For this review, take the finished solid that the model builds, in its own axes (mm). A direction names the side the tool comes from. Round coordinates to 2 decimals unless told otherwise and drop trailing zeros. Write each loop counter-clockwise with the first axis right and the second up, starting at its lowest first coordinate (ties: lowest second). Pieces come first, ordered by that corner, then holes. Notation, with made-up numbers: (85.25, 6.25) -> (123.25, 6.25) arc R19 cw to (123.25, 15.25) -> close; hole circle Ø6 at (-25, 18.5). An arc over 180 degrees is marked (long way). Write item = value, one per line. Start each with the question number.
```python
from build123d import *

# Parameters (mm, degrees)
CUT_EXTRUDE1_DEPTH = 2.5


with BuildPart() as part:
    # Sketch1 → Revolve1 (revolve)
    with BuildSketch(Plane(origin=(0, 0, 0), x_dir=(0, 0, -1), z_dir=(1, 0, 0)), mode=Mode.PRIVATE) as revolve1_sk:
        with BuildLine():
            Line((-1.633974596, 0), (-2.5, 1.5))
            Line((-2.5, 1.5), (-2.5, 3.8))
            ThreePointArc((-2.5, 3.8), (-2.441421356, 3.941421356), (-2.3, 4))
            Line((-2.3, 4), (-0.833333333, 4))
            Line((-0.833333333, 4), (-0.833333333, 3.6))
            Line((-0.833333333, 3.6), (-0.683333333, 3.6))
            Line((-0.683333333, 3.6), (-0.683333333, 4))
            Line((-0.683333333, 4), (0, 4))
            Line((0, 4), (0, 2.0095))
            Line((0, 2.0095), (0.4905, 2.5))
            Line((0.4905, 2.5), (3.3095, 2.5))
            Line((3.3095, 2.5), (3.8, 2.0095))
            Line((3.8, 2.0095), (3.8, 0))
            Line((3.8, 0), (-1.633974596, 0))
        make_face()
    revolve(revolve1_sk.sketch.rotate(Axis((0, 0, -3.8), (0, 0, 1)), 180), axis=Axis((0, 0, -3.8), (0, 0, 1)))

    # Sketch2 → Cut-Extrude1 (cut)
    with BuildSketch(Plane.XY.offset(2.5)):
        Polygon((-1.25, -0.721687836), (0, -1.443375673), (1.25, -0.721687836), (1.25, 0.721687836), (0, 1.443375673), (-1.25, 0.721687836), align=None)
    extrude(amount=-CUT_EXTRUDE1_DEPTH, mode=Mode.SUBTRACT)


solid = part.part
```
1. Machinability: for faces 1 (the cylindrical face through (-3.905, 0.867, 0.337)), 2 (the cylindrical face through (0.1, 2.5, -1.9)), 3 (the flat face through (-0.63, -1.08, 1.25)), which of the approach directions +Z, -Z, +X, -X, +Y, -Y give a long, thin tool a straight path to every point of the face, cutting with its end or side? Answer none if there is none.
2. Consider section B-B, the plane z = 1.25. Give the boundary of the cut face in (x, y), then the cut area to 3 significant figures.
3. Wall thickness on L1, parallel to Z at x = 2, y = 2.5; L2, parallel to Z at x = 0.25, y = 2.25; L3, parallel to Z at x = -2.25, y = -1: over which ranges is each line inside the solid? List them lowest first. Write a range as from..to.
4. Consider section A-A, the plane y = 0. Give the boundary of the cut face in (x, z), then the cut area to 3 significant figures.
5. Clearance check with flat-ended pins moving along their axes: pin 1 Ø3 at (x, y) = (2.5, 3) entering from -Z; pin 2 Ø1.5 at (x, z) = (-2.5, -1) entering from -Y; pin 3 Ø0.8 at (x, y) = (-0.5, 0) entering from +Z. State where each tip first meets the part, or that it passes through.
6. Consider section C-C, the plane z = -2.5. Give the boundary of the cut face in (x, y).
Outcome:
q1.face_1 = +Z, -Z
q1.face_2 = -Z
q1.face_3 = +Z
q2.outline = circle Ø8 at (0, 0); hole (-1.25, -0.72) -> (0, -1.44) -> (1.25, -0.72) -> (1.25, 0.72) -> (0, 1.44) -> (-1.25, 0.72) -> close
q2.area = 44.9 mm2
q3.L1 = 0..2.5
q3.L2 = -3.55..-0.25, 0..2.5
q3.L3 = -3.35..-0.45, 0..2.5
q4.outline = (-4, 0) -> (-2.01, 0) -> (-2.5, -0.49) -> (-2.5, -3.31) -> (-2.01, -3.8) -> (2.01, -3.8) -> (2.5, -3.31) -> (2.5, -0.49) -> (2.01, 0) -> (4, 0) -> (4, 0.68) -> (3.6, 0.68) -> (3.6, 0.83) -> (4, 0.83) -> (4, 2.3) arc R0.2 ccw to (3.8, 2.5) -> (1.5, 2.5) -> (1.25, 2.36) -> (1.25, 0) -> (-1.25, 0) -> (-1.25, 2.36) -> (-1.5, 2.5) -> (-3.8, 2.5) arc R0.2 ccw to (-4, 2.3) -> (-4, 0.83) -> (-3.6, 0.83) -> (-3.6, 0.68) -> (-4, 0.68) -> close
q4.area = 32.1 mm2
q5.pin_1 = -3.4
q5.pin_2 = -1.79
q5.pin_3 = 0
q6.outline = circle Ø5 at (0, 0)
